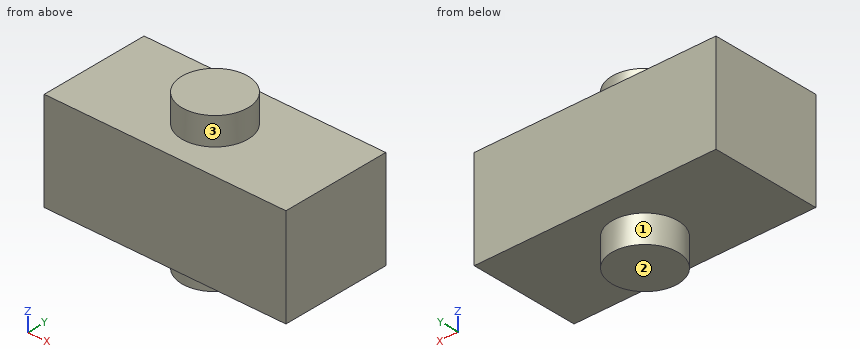
from build123d import *

# Parameters (mm, degrees)
SKETCH_1_W      = 44
SKETCH_1_H      = 20
EXTRUDE_1_DEPTH = 9
SKETCH_2_R      = 6
EXTRUDE_2_DEPTH = 14


with BuildPart() as part:
    # 草图1 → 凸台-拉伸1 (new, symmetric)
    with BuildSketch(Plane.XY):
        Rectangle(SKETCH_1_W, SKETCH_1_H)
    extrude(amount=EXTRUDE_1_DEPTH, both=True)

    # 草图2 → 凸台-拉伸2 (add, symmetric)
    with BuildSketch(Plane.XY):
        Circle(SKETCH_2_R)
    extrude(amount=EXTRUDE_2_DEPTH, both=True)


solid = part.part
Read the model definition and answer for the solid it produces. Units are mm, in the model's axes. Face numbers are marked on the shaded views. A direction names the side the tool comes from. Coordinates: 2 decimals unless noted, no trailing zeros. Write each loop counter-clockwise with the first axis right and the second up, starting at its lowest first coordinate (ties: lowest second). Pieces come first, ordered by that corner, then holes. Notation, with made-up numbers: (19.5, -9.75) -> (28.5, -9.75) arc R30 cw to (28.5, 22.25) -> close; hole circle Ø9 at (4.25, 28). An arc over 180 degrees is marked (long way). Return JSON: item names as keys, results as strings.
(1) Each of these flat-tipped pins is pushed along its axis until it touches: P1, Ø4, axis at x = -6, y = -5, coming from the +Z side; P2, Ø4, axis at x = -6.5, y = 6, coming from the +Z side; P3, Ø1, axis at x = -14.5, y = 3.5, coming from the -Z side. Where does it stop, or does it pass through?
Answers below:
{"P1": "z = 14", "P2": "z = 9", "P3": "z = -9"}
(2) The part is cut by section D-D on x = 15. Give the vertices of the cut face in (y, z).
Answers below:
{"outline": "(-10, -9) -> (10, -9) -> (10, 9) -> (-10, 9) -> close"}
(3) The part is cut by section B-B on y = 0. Give the vertices of the cut face in (x, z).
Answers below:
{"outline": "(-22, -9) -> (-6, -9) -> (-6, -14) -> (6, -14) -> (6, -9) -> (22, -9) -> (22, 9) -> (6, 9) -> (6, 14) -> (-6, 14) -> (-6, 9) -> (-22, 9) -> close"}
(4) The part is cut by section C-C on z = -10.5. Give the vertices of the cut face in (x, y), then the cut area to 3 significant figures.
Answers below:
{"outline": "circle Ø12 at (0, 0)", "area": "113 mm^2"}
(5) Consider line 1 along Z through (x, y) = (20, 0); line 2 along Y through (x, z) = (1, 9.75); line 3 along Y through (x, z) = (-2, 9.75). Determine where each line is inside the solid, lowest interval first. Write a range as from..to.
Answers below:
{"line 1": "-9..9", "line 2": "-5.92..5.92", "line 3": "-5.66..5.66"}
(6) The part is cut by section A-A on x = 0. Give the vertices of the cut face in (y, z), then the cut area to 3 significant figures.
Answers below:
{"outline": "(-10, -9) -> (-6, -9) -> (-6, -14) -> (6, -14) -> (6, -9) -> (10, -9) -> (10, 9) -> (6, 9) -> (6, 14) -> (-6, 14) -> (-6, 9) -> (-10, 9) -> close", "area": "480 mm^2"}
(7) Which of the six approach directions +Z, -Z, +X, -X, +Y, -Y give full straight-line access (tool end or side, diameter ignored) to the marked faces 1, 2 and 3?
Answers below:
{"face 1": "-Z", "face 2": "-Z, +X, -X, +Y, -Y", "face 3": "+Z"}
